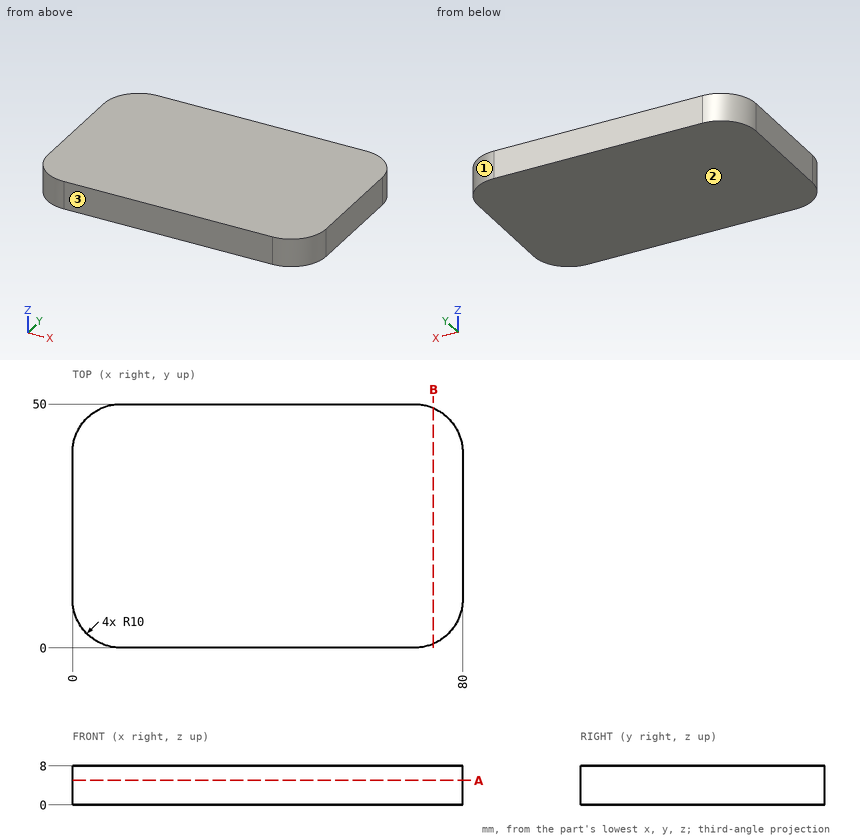
Design review of the part shown in the three views and the two pictorial views. Dimensions are in mm from the part's minimum x, y and z. Round coordinates to 2 decimals unless told otherwise and drop trailing zeros. Loops run counter-clockwise (first coordinate to the right, second up) from the corner with the lowest first, then second, coordinate; pieces in that order, holes last. Notation, with made-up numbers: (-30, 31) -> (-11, 31) arc R26 ccw to (-11, 70) -> close; hole circle Ø8 at (61.5, 85). An arc over 180 degrees is marked (long way). Return JSON: item names as keys, results as strings.
(1) The part is to be moulded in two halves that separate along Y. For the marked faces 1, 2 and 3, say which applies: released by +Y, released by -Y, zero draft, split by the parting line, or undercut.
Solved:
{"face 1": "released by +Y", "face 2": "zero draft", "face 3": "released by -Y"}
(2) For line 1 (X direction, y = 40.5, z = 4.25); line 2 (X direction, y = 7.5, z = 3); line 3 (Y direction, x = 4, z = 0.5), list the stretches that pass through material, from the lowest coordinate up.
Solved:
{"line 1": "0.01 to 79.99", "line 2": "0.32 to 79.68", "line 3": "2 to 48"}
(3) Add section A-A on z = 5. Write out the cut boundary in (x, y).
Solved:
{"outline": "(0, 10) arc R10 ccw to (10, 0) -> (70, 0) arc R10 ccw to (80, 10) -> (80, 40) arc R10 ccw to (70, 50) -> (10, 50) arc R10 ccw to (0, 40) -> close"}
(4) Add section B-B on x = 74. Write out the cut boundary in (y, z).
Solved:
{"outline": "(0.83, 0) -> (49.17, 0) -> (49.17, 8) -> (0.83, 8) -> close"}
